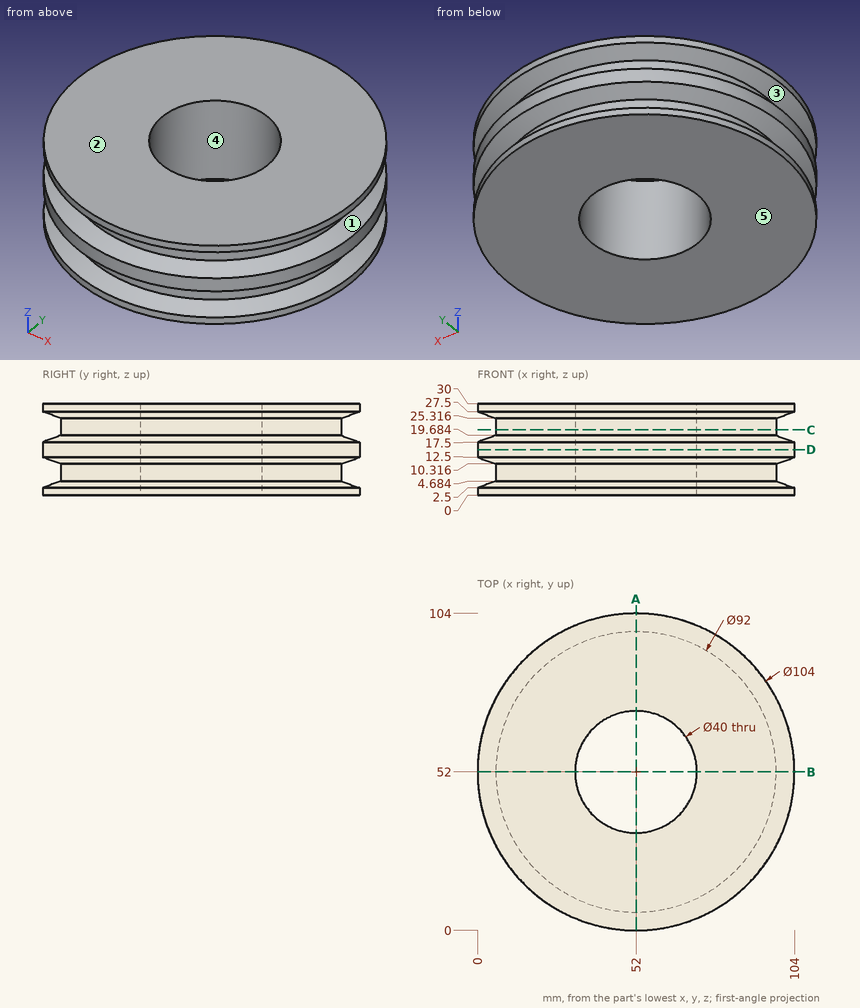
Source: three-view drawing plus pictorial views. Frame: mm from the lowest corner of the part. A direction names the side the tool comes from. Give positions to 0.01 mm unless a question says otherwise; leave off trailing zeros. Loops run counter-clockwise (first coordinate to the right, second up) from the corner with the lowest first, then second, coordinate; pieces in that order, holes last. Notation, with made-up numbers: M 8,43.5 L 25,43.5 A5 cw 25,48.5 Z; hole C 51,-10.5 d11. An arc over 180 degrees is marked long. Put each result on its own line as item: value.
Q1. Reachability of the marked faces 1 and 2 from +Z, -Z, +X, -X, +Y, -Y: full face, straight path, thin tool, end or side. Return the list, or none.
Response values:
face 1: none
face 2: +Z, +X, -X, +Y, -Y
Q2. Mould query, pull axis X, two halves, no side actions, for the marked faces 3, 4 and 5. Classes: released by +X, released by -X, zero draft, split by the parting line, or undercut.
Response values:
face 3: split by the parting line
face 4: undercut
face 5: zero draft
Q3. Pin query (flat end, axial travel): P1, Ø12, axis at x = 90.5, z = 13.5, coming from the +Y side; P2, Ø12, axis at y = 33, z = 9.5, coming from the -X side. Return the tip coordinate at first contact, or that it passes through.
Response values:
P1: stops at y = 92.59
P2: stops at x = 1.87
Q4. Section C-C (z = 21.5). Return the cut outline in (x, y).
Response values:
outline: C 52,52 d92; hole C 52,52 d40
Q5. Line query: probe 1 along Y at (x, z) = (52, 23.25); probe 2 along Y at (x, z) = (52, 14.25); probe 3 along X at (y, z) = (70.5, 7.25) (1 decimal). Output: solid intervals per line, ascending. Write a range as [from, to].
Response values:
probe 1: y = [6, 32], [72, 98]
probe 2: y = [0, 32], [72, 104]
probe 3: x = [9.9, 44.4], [59.6, 94.1]
Q6. Section A-A (x = 52). Return the cut outline in (y, z).
Response values:
outline: M 0,0 L 32,0 L 32,30 L 0,30 L 0,27.5 L 6,25.32 L 6,19.68 L 0,17.5 L 0,12.5 L 6,10.32 L 6,4.68 L 0,2.5 Z; M 72,0 L 104,0 L 104,2.5 L 98,4.68 L 98,10.32 L 104,12.5 L 104,17.5 L 98,19.68 L 98,25.32 L 104,27.5 L 104,30 L 72,30 Z
Q7. Section D-D (z = 15). Return the cut outline in (x, y), and give its area (3 significant figures).
Response values:
outline: C 52,52 d104; hole C 52,52 d40
area: 7,240 mm²
